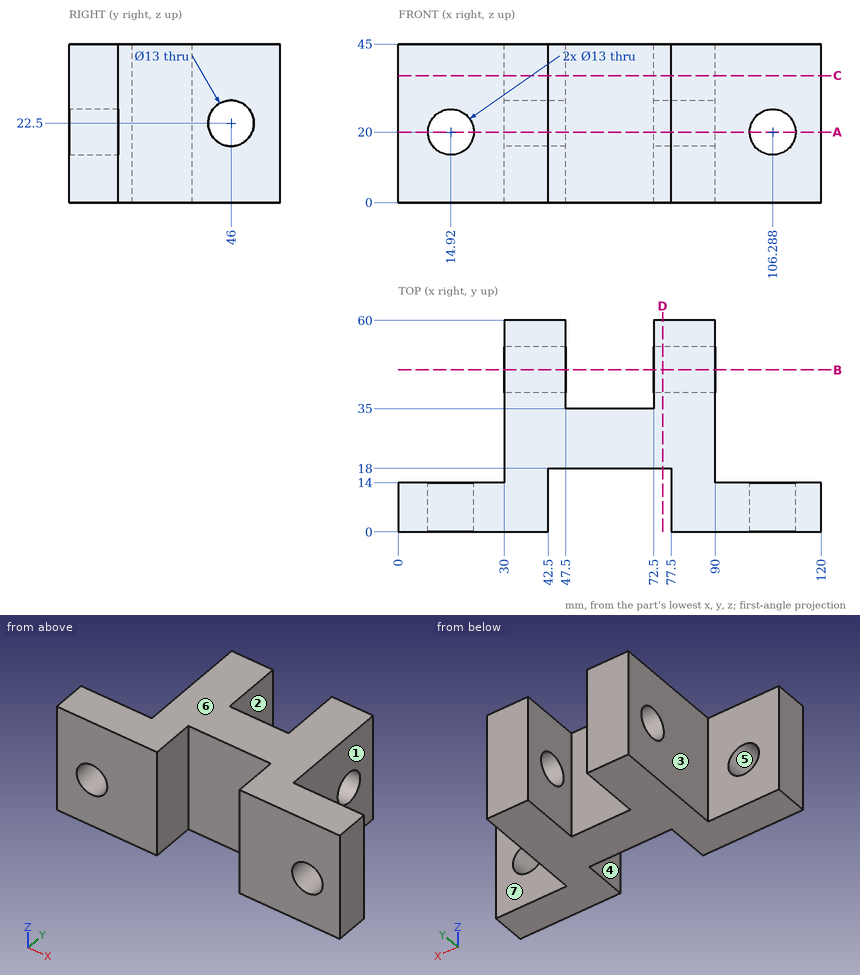
Part print with two shaded views. Sizes in mm from the minimum x, y, z corner. A direction names the side the tool comes from. Round coordinates to 2 decimals unless told otherwise and drop trailing zeros. Write each loop counter-clockwise with the first axis right and the second up, starting at its lowest first coordinate (ties: lowest second). Pieces come first, ordered by that corner, then holes. Notation, with made-up numbers: M 11,7 L 20,7 A36 cw 20,45 Z; hole C 81,-5 d6. An arc over 180 degrees is marked long. Answer as CSV lines item,"result". Start each with the question number.
1) Drill centre lines: L1, parallel to X at y = 7, z = 20; L2, parallel to X at y = 51, z = 33; L3, parallel to Y at x = 78.25, z = 22.5. Where is each one in solid material? Low to high.
2) Band-saw the part on D-D (x = 75). List the corners of the cut face in (y, z), then the cut area to 3 significant figures.
3) Mould opens along Z. For the marked faces 5, 6 and 7 say: +Z half, -Z half, draft (parallel to the pull), parting line (faces both ways), or undercut.
4) Band-saw the part on B-B (y = 46). List the corners of the cut face in (x, z).
5) Band-saw the part on C-C (z = 36). List the corners of the cut face in (x, y), then the cut area to 4 significant figures.
6) Which spindle directions (+Z, -Z, +X, -X, +Y, -Y) get a long thin tool onto all of the face, cutting with end or side? Do the marked faces 1, 2, 3 and 4. Say none if no direction does.
7) Drop flat-ended pins along their axis: pin 1 (17 mm diameter, centred on y = 46, z = 22.5, fed in from +X); pin 2 (10.5 mm diameter, centred on x = 51.5, z = 24.5, fed in from -Y); pin 3 (4 mm diameter, centred on y = 42.5, z = 29.5, fed in from -X); pin 4 (4 mm diameter, centred on x = 37.5, y = 49.5, fed in from -Z). Give the stop position or say it passes through.
8) Band-saw the part on A-A (z = 20). Count the separate pieces of the cut face and the enclosed holes in it, then the cut area to 3 significant figures.
Worked out:
1,L1,"0 to 8.42, 21.42 to 42.5, 77.5 to 99.79, 112.79 to 120"
1,L2,"30 to 47.5, 72.5 to 90"
1,L3,"0 to 39.5, 52.5 to 60"
2,outline,"M 18,0 L 60,0 L 60,45 L 18,45 Z; hole C 46,22.5 d13"
2,area,"1,760 mm²"
3,face 5,"undercut"
3,face 6,"+Z half"
3,face 7,"draft"
4,outline,"M 30,0 L 47.5,0 L 47.5,16 L 30,16 Z; M 30,29 L 47.5,29 L 47.5,45 L 30,45 Z; M 72.5,0 L 90,0 L 90,16 L 72.5,16 Z; M 72.5,29 L 90,29 L 90,45 L 72.5,45 Z"
5,outline,"M 0,0 L 42.5,0 L 42.5,18 L 77.5,18 L 77.5,0 L 120,0 L 120,14 L 90,14 L 90,60 L 72.5,60 L 72.5,35 L 47.5,35 L 47.5,60 L 30,60 L 30,14 L 0,14 Z"
5,area,"3,185 mm²"
6,face 1,"+Z, -Z, +X, +Y"
6,face 2,"+Z, -Z, +Y"
6,face 3,"+Z, -Z, -X, +Y"
6,face 4,"+Z, -Z, -Y"
7,pin 1,"x = 90"
7,pin 2,"y = 18"
7,pin 3,"x = 30"
7,pin 4,"z = 0"
8,separate pieces,"5"
8,enclosed holes,"0"
8,area,"2,400 mm²"
